```python
from build123d import *

# Parameters (mm, degrees)
SKETCH_1_W                = 45
SKETCH_1_H                = 70
EXTRUDE_1_DEPTH           = 8.5
SKETCH_2_W                = 42.5
SKETCH_2_H                = 70
CUT_EXTRUDE_1_DEPTH       = 2
HOLE_WIZARD_1_D           = 5.5
HOLE_WIZARD_1_CBORE_D     = 10
HOLE_WIZARD_1_CBORE_DEPTH = 7
HOLE_WIZARD_18_0_18_1_D   = 18
HOLE_WIZARD_M3_1_D        = 2.5
HOLE_WIZARD_M3_1_DEPTH    = 8.5
HOLE_WIZARD_M3_1_TIP      = 0.751075774


with BuildPart() as part:
    # 草图1 → 凸台-拉伸1 (new, symmetric)
    with BuildSketch(Plane(origin=(0, 0, 0), x_dir=(1, 0, 0), z_dir=(0, 1, 0))):
        Rectangle(SKETCH_1_W, SKETCH_1_H)
    extrude(amount=EXTRUDE_1_DEPTH, both=True)

    # 草图2 → 切除-拉伸1 (cut)
    with BuildSketch(Plane.XZ.offset(8.5)):
        with Locations((1.25, 0)):
            Rectangle(SKETCH_2_W, SKETCH_2_H)
    extrude(amount=-CUT_EXTRUDE_1_DEPTH, mode=Mode.SUBTRACT)

    # 打孔尺寸(%根据)内六角圆柱头螺钉的类型1 (through all)
    with Locations(Plane(origin=(0, 8.5, 0), x_dir=(1, 0, 0), z_dir=(0, 1, 0))):
        with Locations((-12.5, -25), (-12.5, 25), (12.5, 25), (12.5, -25)):
            CounterBoreHole(HOLE_WIZARD_1_D / 2, HOLE_WIZARD_1_CBORE_D / 2, HOLE_WIZARD_1_CBORE_DEPTH)

    # Ø18.0 (18) 直径孔1 (through all)
    with Locations(Plane(origin=(0, 8.5, 0), x_dir=(1, 0, 0), z_dir=(0, 1, 0))):
        with Locations((0, 0)):
            Hole(HOLE_WIZARD_18_0_18_1_D / 2)

    # M3 螺纹孔1
    with Locations(Plane(origin=(22.5, 0, 0), x_dir=(0, 0, -1), z_dir=(1, 0, 0))):
        with Locations((7.5, -1.5), (-7.5, -1.5)):
            Hole(HOLE_WIZARD_M3_1_D / 2, depth=HOLE_WIZARD_M3_1_DEPTH)
            with Locations((0, 0, -(HOLE_WIZARD_M3_1_DEPTH + HOLE_WIZARD_M3_1_TIP / 2))):  # 118° drill point
                Cone(0, HOLE_WIZARD_M3_1_D / 2, HOLE_WIZARD_M3_1_TIP, mode=Mode.SUBTRACT)


solid = part.part
```
Geometry check sheet. Reference: the model listing, model coordinates, mm. A direction names the side the tool comes from. Coordinates: 2 decimals unless noted, no trailing zeros. Loops run counter-clockwise (first coordinate to the right, second up) from the corner with the lowest first, then second, coordinate; pieces in that order, holes last.
Item 1: Access from +Z, -Z, +X, -X, +Y, -Y to the whole of each face (thin tool, end or side, straight path). Record for faces 4 (the face through (0, 0, 35)), 5 (the face through (-22.5, 0, 0)), 6 (the face through (6, -6.5, -7)), 7 (the face through (-10, 1.5, -23)), 8 (the face through (18.19, -1.45, 6.25)).
Item 2: Sectioned sample at C-C, the plane y = -3.5. Record the boundary of the cut face in (x, z), then the cut area to 3 significant figures.
Item 3: Sectioned sample at A-A, the plane x = 12.5. Record the boundary of the cut face in (y, z), then the cut area to 3 significant figures.
Item 4: Sectioned sample at B-B, the plane z = 25. Record the boundary of the cut face in (x, y), then the cut area to 3 significant figures.
Item 5: Thickness scan on line 1 (Z direction, x = 12.5, y = 4.75); line 2 (X direction, y = 6.25, z = 25); line 3 (X direction, y = 2, z = -27). Record the ranges inside material, lowest first.
Item 6: Sectioned sample at D-D, the plane z = 0. Record the boundary of the cut face in (x, y), then the cut area to 3 significant figures.
Item 7: Release check for a two-part mould opening along Y. For faces 1 (the face through (14.807, 5.049, -20.564)), 2 (the face through (18.19, -1.45, -8.75)), 3 (the face through (-10, 1.5, 27)) record: released by +Y, released by -Y, zero draft, split by the parting line, or undercut.
Item 8: Go/stop test with flat-tipped pins: pin 1 Ø4.5 at (x, z) = (12.5, -25) entering from +Y; pin 2 Ø1.6 at (y, z) = (-7.5, 2) entering from +X; pin 3 Ø13 at (x, z) = (-2.5, 4.5) entering from -Y; pin 4 Ø3 at (x, z) = (-14.5, -25) entering from +Y. Record where each tip stops, or that it passes through.
Check result:
1. face 4: +Z, +X, -X, +Y, -Y
1. face 5: +Z, -Z, -X, +Y, -Y
1. face 6: +Z, -Z, +X, -Y
1. face 7: +Y
1. face 8: +X
2. outline: (-22.5, -35) - (22.5, -35) - (22.5, 35) - (-22.5, 35) - close; hole circle Ø5.5 at (-12.5, -25); hole circle Ø5.5 at (-12.5, 25); hole circle Ø18 at (0, 0); hole circle Ø5.5 at (12.5, -25); hole circle Ø5.5 at (12.5, 25)
2. area: 2,800 mm2
3. outline: (-6.5, -35) - (8.5, -35) - (8.5, -30) - (1.5, -30) - (1.5, -27.75) - (-6.5, -27.75) - close; (-6.5, -22.25) - (1.5, -22.25) - (1.5, -20) - (8.5, -20) - (8.5, 20) - (1.5, 20) - (1.5, 22.25) - (-6.5, 22.25) - close; (-6.5, 27.75) - (1.5, 27.75) - (1.5, 30) - (8.5, 30) - (8.5, 35) - (-6.5, 35) - close
3. area: 822 mm2
4. outline: (-22.5, -8.5) - (-20, -8.5) - (-20, -6.5) - (-15.25, -6.5) - (-15.25, 1.5) - (-17.5, 1.5) - (-17.5, 8.5) - (-22.5, 8.5) - close; (-9.75, -6.5) - (9.75, -6.5) - (9.75, 1.5) - (7.5, 1.5) - (7.5, 8.5) - (-7.5, 8.5) - (-7.5, 1.5) - (-9.75, 1.5) - close; (15.25, -6.5) - (22.5, -6.5) - (22.5, 8.5) - (17.5, 8.5) - (17.5, 1.5) - (15.25, 1.5) - close
4. area: 452 mm2
5. line 1: z = -35 to -30, -20 to 20, 30 to 35
5. line 2: x = -22.5 to -17.5, -7.5 to 7.5, 17.5 to 22.5
5. line 3: x = -22.5 to -17.08, -7.92 to 7.92, 17.08 to 22.5
6. outline: (-22.5, -8.5) - (-20, -8.5) - (-20, -6.5) - (-9, -6.5) - (-9, 8.5) - (-22.5, 8.5) - close; (9, -6.5) - (22.5, -6.5) - (22.5, 8.5) - (9, 8.5) - close
6. area: 410 mm2
7. face 1: zero draft
7. face 2: undercut
7. face 3: released by +Y
8. pin 1: passes through
8. pin 2: stops at x = -20
8. pin 3: stops at y = -6.5
8. pin 4: stops at y = 1.5
